from build123d import *

# Parameters (mm, degrees)
SKETCH1_W                 = 125
SKETCH1_H                 = 60
BOSS_EXTRUDE1_DEPTH       = 6
M6_TAPPED_HOLE1_D         = 5
M4_TAPPED_HOLE1_D         = 3.3
SKETCH8_R                 = 4.5
CUT_EXTRUDE1_DEPTH        = 2
BLIND_PIN_HOLE1_SIZE_MM_D = 5
CHAMFER1_SIZE             = 1


with BuildPart() as part:
    # Sketch1 → Boss-Extrude1 (new, symmetric)
    with BuildSketch(Plane.XY):
        Rectangle(SKETCH1_W, SKETCH1_H)
    extrude(amount=BOSS_EXTRUDE1_DEPTH, both=True)

    # M6 Tapped Hole1 (through all)
    with Locations(Plane(origin=(0, 0, -6), x_dir=(-1, 0, 0), z_dir=(0, 0, -1))):
        with Locations((5, 24), (5, -24), (-55, -24), (-55, 24)):
            Hole(M6_TAPPED_HOLE1_D / 2)

    # M4 Tapped Hole1 (through all)
    with Locations(Plane.XY.offset(6)):
        with Locations((-1.5, 9.5), (-1.5, -9.5), (-41.5, -9.5), (-41.5, 9.5)):
            Hole(M4_TAPPED_HOLE1_D / 2)

    # Sketch8 → Cut-Extrude1 (cut)
    with BuildSketch(Plane.XY.offset(6)):
        with Locations((-41.5, 9.5)):
            Circle(SKETCH8_R)
        with Locations((-41.5, -9.5)):
            Circle(SKETCH8_R)
    extrude(amount=-CUT_EXTRUDE1_DEPTH, mode=Mode.SUBTRACT)

    # Blind Pin Hole1 (size mm) (through all)
    with Locations(Plane.XY.offset(6)):
        with Locations((10, 24), (40, 24), (10, -24), (40, -24)):
            Hole(BLIND_PIN_HOLE1_SIZE_MM_D / 2)

    # Chamfer1
    chamfer1_edges = [part.edges().sort_by_distance(p)[0] for p in [
        (62.5, -30, 0),
        (-62.5, -30, 0),
        (-62.5, 30, 0),
        (62.5, 30, 0),
    ]]
    chamfer(chamfer1_edges, length=CHAMFER1_SIZE)


solid = part.part
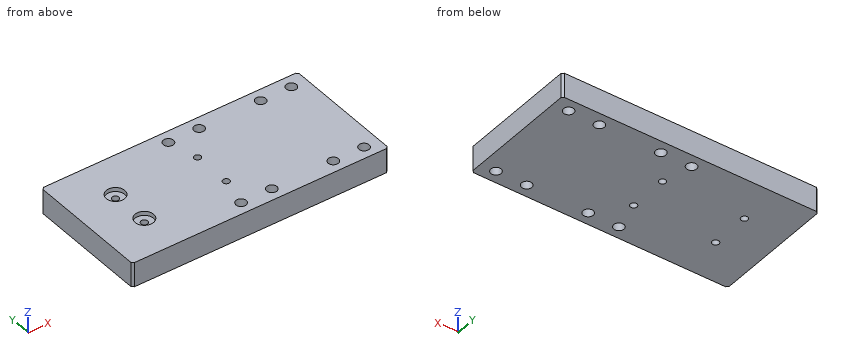
Design review of the part built by this model. Coordinates are the model's own, in mm. Round coordinates to 2 decimals unless told otherwise and drop trailing zeros. Write each loop counter-clockwise with the first axis right and the second up, starting at its lowest first coordinate (ties: lowest second). Pieces come first, ordered by that corner, then holes.
Item 1: Consider section B-B on x = -41.5. Give the boundary of the cut face in (y, z), and give its area (3 significant figures).
Item 2: Consider section D-D on z = -0.75. Count the separate pieces of the cut face and the enclosed holes in it, and give its area (3 significant figures).
Item 3: For pin 1 Ø4.5 at (x, y) = (-5, 24) entering from +Z; pin 2 Ø8 at (x, y) = (-41.5, 9.5) entering from +Z, all flat-tipped, find the tip position at first contact; note any pin that passes through.
Item 4: Consider section C-C on y = -24. Give the boundary of the cut face in (x, z).
Item 5: Consider section A-A on y = 9.5. Give the boundary of the cut face in (x, z), and give its area (3 significant figures).
Item 6: Wall thickness on L1, parallel to Y at x = -41.5, z = -1.75; L2, parallel to Y at x = 10, z = 3.5; L3, parallel to X at y = -10.5, z = -2.75: over which ranges is each line inside the solid? List them lowest first.
Check values:
1. outline: (-30, -6) - (-11.15, -6) - (-11.15, 4) - (-14, 4) - (-14, 6) - (-30, 6) - close; (-7.85, -6) - (7.85, -6) - (7.85, 4) - (5, 4) - (5, 6) - (-5, 6) - (-5, 4) - (-7.85, 4) - close; (11.15, -6) - (30, -6) - (30, 6) - (14, 6) - (14, 4) - (11.15, 4) - close
1. area: 618 mm2
2. separate pieces: 1
2. enclosed holes: 12
2. area: 7,310 mm2
3. pin 1: passes through
3. pin 2: stops at z = 4
4. outline: (-62.5, -6) - (-7.5, -6) - (-7.5, 6) - (-62.5, 6) - close; (-2.5, -6) - (7.5, -6) - (7.5, 6) - (-2.5, 6) - close; (12.5, -6) - (37.5, -6) - (37.5, 6) - (12.5, 6) - close; (42.5, -6) - (52.5, -6) - (52.5, 6) - (42.5, 6) - close; (57.5, -6) - (62.5, -6) - (62.5, 6) - (57.5, 6) - close
5. outline: (-62.5, -6) - (-43.15, -6) - (-43.15, 4) - (-46, 4) - (-46, 6) - (-62.5, 6) - close; (-39.85, -6) - (-3.15, -6) - (-3.15, 6) - (-37, 6) - (-37, 4) - (-39.85, 4) - close; (0.15, -6) - (62.5, -6) - (62.5, 6) - (0.15, 6) - close
5. area: 1,410 mm2
6. L1: y = -30 to -11.15, -7.85 to 7.85, 11.15 to 30
6. L2: y = -30 to -26.5, -21.5 to 21.5, 26.5 to 30
6. L3: x = -62.5 to -42.81, -40.19 to -2.81, -0.19 to 62.5
